from build123d import *

# Parameters (mm, degrees)
SKETCH1_R           = 12
SKETCH1_R_2         = 4
BOSS_EXTRUDE1_DEPTH = 51
SKETCH2_R           = 8
CUT_EXTRUDE1_DEPTH  = 47
BOSS_EXTRUDE2_START = -6
SKETCH3_R           = 21
SKETCH3_R_2         = 12
BOSS_EXTRUDE2_DEPTH = 6
SKETCH4_R           = 2
CUT_EXTRUDE2_DEPTH  = 6
SKETCH5_R           = 3
CUT_EXTRUDE3_DEPTH  = 3
CIRPATTERN1_COUNT   = 4
CHAMFER1_SIZE       = 1


with BuildPart() as part:
    # Sketch1 → Boss-Extrude1 (new body)
    with BuildSketch(Plane(origin=(0, 0, 0), x_dir=(1, 0, 0), z_dir=(0, 1, 0))):
        with Locations(Location((0, 0, 0), (0, 0, 270))):
            Circle(SKETCH1_R)
        with Locations(Location((0, 0, 0), (0, 0, 270))):
            Circle(SKETCH1_R_2, mode=Mode.SUBTRACT)
    extrude(amount=BOSS_EXTRUDE1_DEPTH)

    # Sketch2 → Cut-Extrude1 (cut)
    with BuildSketch(Plane.XZ):
        with Locations(Location((0, 0, 0), (0, 0, 270))):
            Circle(SKETCH2_R)
    extrude(amount=-CUT_EXTRUDE1_DEPTH, mode=Mode.SUBTRACT)

    # Sketch3 → Boss-Extrude2 (add)
    with BuildSketch(Plane(origin=(0, 35, 0), x_dir=(-1, 0, 0), z_dir=(0, 1, 0)).offset(BOSS_EXTRUDE2_START)):
        with Locations(Location((0, 0, 0), (0, 0, 90))):
            Circle(SKETCH3_R)
        with Locations(Location((0, 0, 0), (0, 0, 90))):
            Circle(SKETCH3_R_2, mode=Mode.SUBTRACT)
    extrude(amount=BOSS_EXTRUDE2_DEPTH)

    # Sketch4 → Cut-Extrude2 (cut)
    with BuildSketch(Plane(origin=(0, 35, 0), x_dir=(1, 0, 0), z_dir=(0, 1, 0))):
        with Locations(Location((0, 16.5, 0), (0, 0, 270))):
            Circle(SKETCH4_R)
    cut_extrude2 = extrude(amount=-CUT_EXTRUDE2_DEPTH, mode=Mode.SUBTRACT)

    # Sketch5 → Cut-Extrude3 (cut)
    with BuildSketch(Plane(origin=(0, 35, 0), x_dir=(1, 0, 0), z_dir=(0, 1, 0))):
        with Locations(Location((0, 16.5, 0), (0, 0, 270))):
            Circle(SKETCH5_R)
    cut_extrude3 = extrude(amount=-CUT_EXTRUDE3_DEPTH, mode=Mode.SUBTRACT)

    # CirPattern1: Cut-Extrude2, Cut-Extrude3 ×4 about axis
    cirpattern1_axis = Axis((0, 0, 0), (0, 1, 0))
    add([cut_extrude2.rotate(cirpattern1_axis, i * 360 / CIRPATTERN1_COUNT) for i in range(1, CIRPATTERN1_COUNT)], mode=Mode.SUBTRACT)
    add([cut_extrude3.rotate(cirpattern1_axis, i * 360 / CIRPATTERN1_COUNT) for i in range(1, CIRPATTERN1_COUNT)], mode=Mode.SUBTRACT)

    # Chamfer1
    chamfer1_edges = [part.edges().sort_by_distance(p)[0] for p in [
        (0, 35, -21),
        (0, 0, -12),
    ]]
    chamfer(chamfer1_edges, length=CHAMFER1_SIZE)


solid = part.part
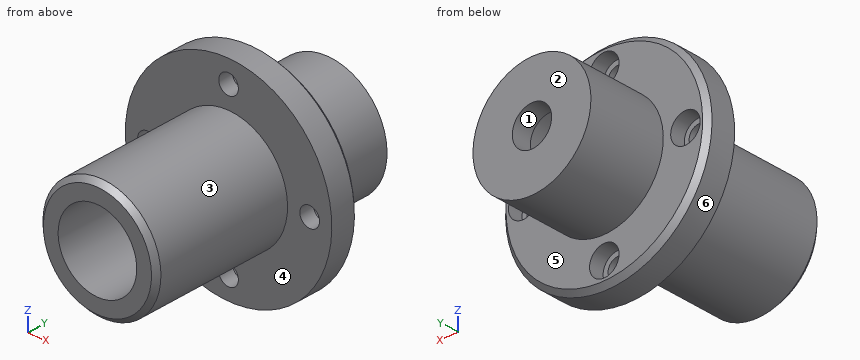
For this review, take the finished solid that the model builds, in its own axes (mm). Face numbers are marked on the shaded views. A direction names the side the tool comes from. Round coordinates to 2 decimals unless told otherwise and drop trailing zeros. Order: outer loops, then holes, each group sorted by start corner. A loop starts at its lowest first (then second) coordinate and runs counter-clockwise, first axis right, second up. Notation, with made-up numbers: M -35,13 L -18,13 A25 cw -18,35 Z; hole C -17,1.5 d10. An arc over 180 degrees is marked long. Use a Markdown table: item, result. Add a question column.
Item 1: Mouldability with a two-part tool opening along Z and no side actions: class the marked faces 1, 2 and 3 as released by +Z, released by -Z, zero draft, split by the parting line, or undercut.
Item 2: Add section B-B, the plane y = 41. Give the boundary of the cut face in (x, z), then the cut area to 3 significant figures.
Item 3: Tool access review of the marked faces 4, 5 and 6: name each direction out of +Z, -Z, +X, -X, +Y, -Y from which nothing blocks a thin tool from reaching the whole face with its end or side.
Item 4: Add section A-A, the plane z = 0. State how many separate pieces and enclosed holes the cut face has, then the cut area to 3 significant figures.
Item 5: To check wall thickness, follow line 1 along X through (y, z) = (50, 0); line 2 along X through (y, z) = (46, 0.5); line 3 along Y through (x, z) = (10.5, 11.5). State the ranges of each line that lie inside material, in increasing order.
Item 6: Insertion check: pin 1 (9.5 mm diameter, centred on x = 0, z = -16.5, fed in from -Y); pin 2 (2 mm diameter, centred on x = -7, y = 29.5, fed in from +Z); pin 3 (6.5 mm diameter, centred on x = -16.5, z = 0, fed in from +Y); pin 4 (10 mm diameter, centred on x = 9, z = 11, fed in from -Y). Each pin has a flat end and moves straight along its axis. Give the tip position at first contact, or say it passes through.
Geometry results:
| question | item | result |
|---|---|---|
| 1 | face 1 | undercut |
| 1 | face 2 | zero draft |
| 1 | face 3 | split by the parting line |
| 2 | outline | C 0,0 d24; hole C 0,0 d16 |
| 2 | area | 251 mm² |
| 3 | face 4 | -Y |
| 3 | face 5 | +Y |
| 3 | face 6 | +Y, -Y |
| 4 | separate pieces | 4 |
| 4 | enclosed holes | 0 |
| 4 | area | 486 mm² |
| 5 | line 1 | x = -12 to -4, 4 to 12 |
| 5 | line 2 | x = -11.99 to -7.98, 7.98 to 11.99 |
| 5 | line 3 | y = 29 to 35 |
| 6 | pin 1 | stops at y = 0.75 |
| 6 | pin 2 | stops at z = 20.12 |
| 6 | pin 3 | stops at y = 35 |
| 6 | pin 4 | stops at y = 0 |
